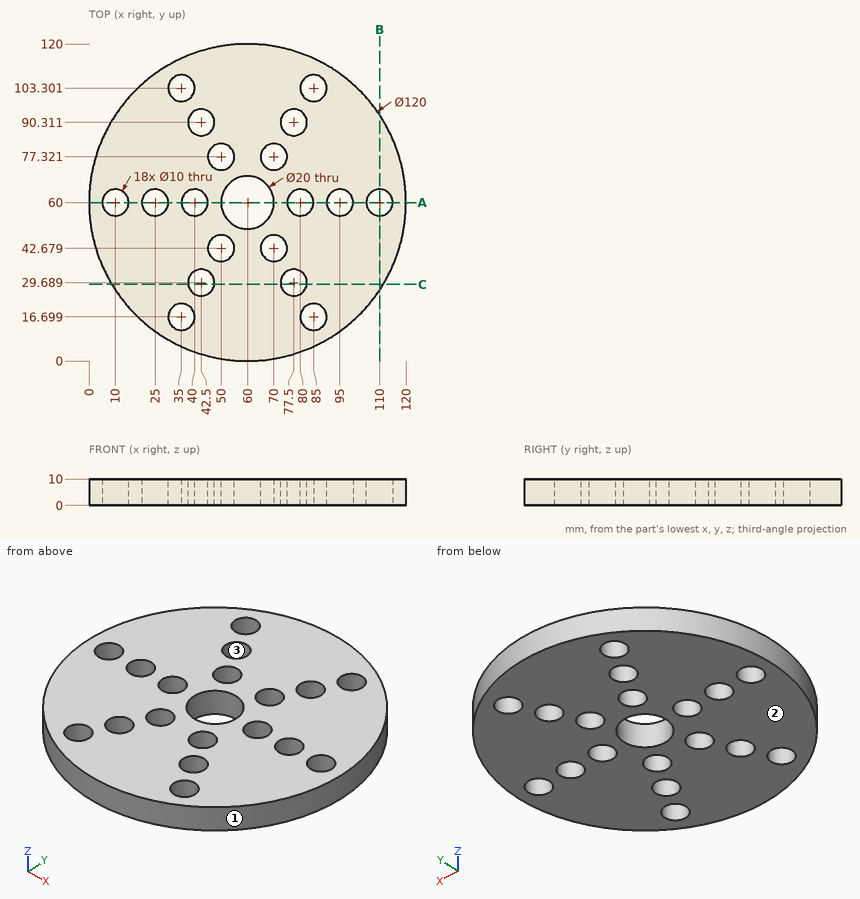
Geometry check sheet. Reference: drawing and pictorial views, mm from the part's lowest x, y, z. Coordinates: 2 decimals unless noted, no trailing zeros. Loops run counter-clockwise (first coordinate to the right, second up) from the corner with the lowest first, then second, coordinate; pieces in that order, holes last.
1) Gauge pin test, flat ends, axial feed: pin 1 (4 mm diameter, centred on y = 83.5, z = 8.5, fed in from +X) (1 decimal); pin 2 (1 mm diameter, centred on y = 36, z = 5.5, fed in from +X); pin 3 (1 mm diameter, centred on y = 46, z = 4.5, fed in from +X). Record the tip position at first contact, or that the pin passes through.
2) Material ranges on probe 1 along X at (y, z) = (43, 4.75); probe 2 along X at (y, z) = (105, 2.5) (1 decimal); probe 3 along Y at (x, z) = (77.5, 7.5), recorded low to high.
3) Sectioned sample at A-A (y = 60). Count the separate pieces of the cut face and the enclosed holes in it, and give its area (3 significant figures).
4) Release check for a two-part mould opening along X. For the marked faces 1, 2 and 3 record: released by +X, released by -X, zero draft, split by the parting line, or undercut.
5) Sectioned sample at C-C (y = 29). Record the boundary of the cut face in (x, z).
6) Sectioned sample at B-B (x = 110). Record the boundary of the cut face in (y, z), and give its area (3 significant figures).
Check sheet entries:
1. pin 1: stops at x = 116
1. pin 2: stops at x = 115.21
1. pin 3: stops at x = 118.46
2. probe 1: x = 2.46 to 45.01, 54.99 to 65.01, 74.99 to 117.54
2. probe 2: x = 20.3 to 30.3, 39.7 to 80.3, 89.7 to 99.7
2. probe 3: y = 2.61 to 24.69, 34.69 to 55.67, 64.33 to 85.31, 95.31 to 117.39
3. separate pieces: 8
3. enclosed holes: 0
3. area: 400 mm2
4. face 1: split by the parting line
4. face 2: zero draft
4. face 3: undercut
5. outline: (8.63, 0) - (37.55, 0) - (37.55, 10) - (8.63, 10) - close; (47.45, 0) - (72.55, 0) - (72.55, 10) - (47.45, 10) - close; (82.45, 0) - (111.37, 0) - (111.37, 10) - (82.45, 10) - close
6. outline: (26.83, 0) - (55, 0) - (55, 10) - (26.83, 10) - close; (65, 0) - (93.17, 0) - (93.17, 10) - (65, 10) - close
6. area: 563 mm2
